from build123d import *

# Parameters (mm, degrees)
SKETCH_1_W          = 300
SKETCH_1_H          = 180
EXTRUDE_1_DEPTH     = 12
SKETCH_2_W          = 300
SKETCH_2_H          = 43
SKETCH_2_H_2        = 51
CUT_EXTRUDE_1_DEPTH = 1.5
SKETCH_3_W          = 20
SKETCH_3_H          = 5
CUT_EXTRUDE_2_DEPTH = 1.5
CUT_EXTRUDE_3_REACH = 177.243


with BuildPart() as part:
    # 草图1 → 凸台-拉伸1 (new body)
    with BuildSketch(Plane.XY):
        Rectangle(SKETCH_1_W, SKETCH_1_H)
    extrude(amount=EXTRUDE_1_DEPTH)

    # 草图2 → 切除-拉伸1 (cut)
    with BuildSketch(Plane(origin=(0, 0, 0), x_dir=(-1, 0, 0), z_dir=(0, 0, -1))):
        with Locations((0, 63.5)):
            Rectangle(SKETCH_2_W, SKETCH_2_H)
        with Locations((0, -64.5)):
            Rectangle(SKETCH_2_W, SKETCH_2_H_2)
    extrude(amount=-CUT_EXTRUDE_1_DEPTH, mode=Mode.SUBTRACT)

    # 草图3 → 切除-拉伸2 (cut)
    with BuildSketch(Plane(origin=(0, 0, 0), x_dir=(-1, 0, 0), z_dir=(0, 0, -1))):
        with Locations((0, 87.5)):
            Rectangle(SKETCH_3_W, SKETCH_3_H)
    extrude(amount=-CUT_EXTRUDE_2_DEPTH, mode=Mode.SUBTRACT)

    # 草图4 → 切除-拉伸3 (cut, up to next)
    with BuildSketch(Plane(origin=(0, 0, 1.5), x_dir=(-1, 0, 0), z_dir=(0, 0, -1)), mode=Mode.PRIVATE) as cut_extrude_3_sk1:
        with BuildLine():
            Line((-7.5, 83), (-7.5, 86))
            ThreePointArc((-7.5, 86), (-5, 88.5), (-2.5, 86))
            Line((-2.5, 86), (-2.5, 83))
            ThreePointArc((-2.5, 83), (-5, 80.5), (-7.5, 83))
        make_face()
    cut_extrude_3_tool1 = extrude(cut_extrude_3_sk1.sketch, amount=-CUT_EXTRUDE_3_REACH, mode=Mode.PRIVATE) & part.part
    cut_extrude_3 = cut_extrude_3_tool1.solids().sort_by_distance((5, 84.5, 1.5))[0]
    add(cut_extrude_3, mode=Mode.SUBTRACT)

    # 镜向1: 切除-拉伸3 across plane
    add(cut_extrude_3.mirror(Plane(origin=(0, 0, 0), x_dir=(0, 0, 1), z_dir=(1, 0, 0))), mode=Mode.SUBTRACT)


solid = part.part
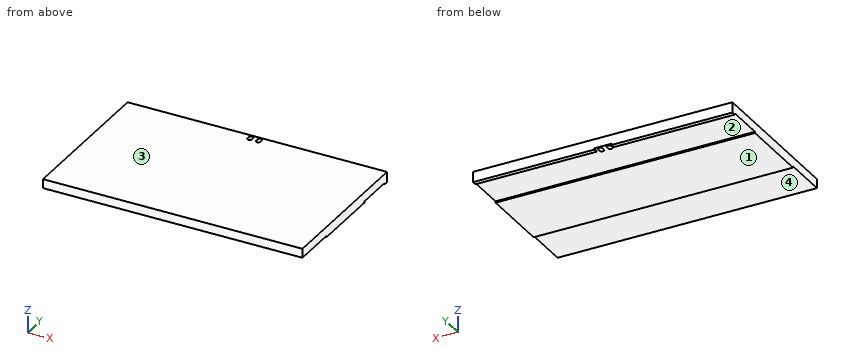
Build history of the part. All positions in model axes, mm. Face numbers are marked on the shaded views. A direction names the side the tool comes from. Round coordinates to 2 decimals unless told otherwise and drop trailing zeros. Write each loop counter-clockwise with the first axis right and the second up, starting at its lowest first coordinate (ties: lowest second). Pieces come first, ordered by that corner, then holes. Notation, with made-up numbers: (63.25, 85) -> (85.25, 85) arc R18 cw to (85.25, 96) -> close; hole circle Ø1 at (34, 72). An arc over 180 degrees is marked (long way). Use one line per item in the form item = value.
Q1. Drill centre lines: L1, parallel to Y at x = -127.5, z = 0.5; L2, parallel to Z at x = 7, y = -45.5. Where is each one in solid material? Low to high.
Conclusion:
L1 = -39 to 42, 85 to 90
L2 = 1.5 to 12
Q2. Band-saw the part on A-A, the plane x = 42.5. Write the cut outline in (y, z).
Conclusion:
outline = (-90, 1.5) -> (-39, 1.5) -> (-39, 0) -> (42, 0) -> (42, 1.5) -> (85, 1.5) -> (85, 0) -> (90, 0) -> (90, 12) -> (-90, 12) -> close
Q3. Band-saw the part on B-B, the plane y = 74. Write the cut outline in (x, z), then the cut area to 3 significant figures.
Conclusion:
outline = (-150, 1.5) -> (150, 1.5) -> (150, 12) -> (-150, 12) -> close
area = 3,150 mm²
Q4. Drop flat-ended pins along their axis: P1, Ø3, axis at x = -97, y = -58, coming from the -Z side; P2, Ø1.2, axis at x = -60, z = 0.5, coming from the -Y side. Give the stop position or say it passes through.
Conclusion:
P1 = 1.5
P2 = -39
Q5. Tool access for the marked faces 3 and 4: list every direction of +Z, -Z, +X, -X, +Y, -Y with a clear straight run to the whole face (end or side of a thin tool).
Conclusion:
face_3 = +Z, +X, -X, +Y, -Y
face_4 = -Z, +X, -X, -Y
Q6. Two-plate mould, pull along Y, no slides. Class the marked faces 1 and 2: released by +Y, released by -Y, zero draft, split by the parting line, or undercut.
Conclusion:
face_1 = zero draft
face_2 = undercut
